```python
from build123d import *

# Parameters (mm, degrees)
BOSS_EXTRUDE1_DEPTH = 48
CHAMFER1_SIZE       = 1
CHAMFER1_SIZE2      = 0.5
CHAMFER2_SIZE       = 0.5
CHAMFER2_SIZE2      = 1.5
CHAMFER3_SIZE       = 0.5
CHAMFER3_SIZE2      = 2.5
CHAMFER4_SIZE       = 2.5
CHAMFER4_SIZE2      = 0.5
CHAMFER5_SIZE       = 4
CHAMFER5_SIZE2      = 3.356398525
CHAMFER6_SIZE       = 4
CHAMFER6_SIZE2      = 3.356398525
FILLET1_R           = 2


with BuildPart() as part:
    # Sketch1 → Boss-Extrude1 (new body)
    with BuildSketch(Plane(origin=(0, 0, 0), x_dir=(1, 0, 0), z_dir=(0, 1, 0))):
        Polygon((-7.5, 2.25), (7.5, 2.25), (7.5, -2.25), (2.45, -2.25), (2.45, -6.75), (2.05, -6.75), (2.05, -3.75), (-2.05, -3.75), (-2.05, -6.75), (-2.45, -6.75), (-2.45, -2.25), (-7.5, -2.25), align=None)
    extrude(amount=BOSS_EXTRUDE1_DEPTH)

    # Chamfer1
    chamfer1_edges = [part.edges().sort_by_distance(p)[0] for p in [
        (-2.05, 24, 3.75),
    ]]
    chamfer1_side = [part.faces().sort_by_distance(p)[0] for p in [
        (-2.05, 24, 5.25),
    ]]
    chamfer(chamfer1_edges, length=CHAMFER1_SIZE, length2=CHAMFER1_SIZE2, reference=chamfer1_side[0])

    # Chamfer2
    chamfer2_edges = [part.edges().sort_by_distance(p)[0] for p in [
        (2.05, 24, 3.75),
    ]]
    chamfer2_side = [part.faces().sort_by_distance(p)[0] for p in [
        (0.25, 24, 3.75),
    ]]
    chamfer(chamfer2_edges, length=CHAMFER2_SIZE, length2=CHAMFER2_SIZE2, reference=chamfer2_side[0])

    # Chamfer3
    chamfer3_edges = [part.edges().sort_by_distance(p)[0] for p in [
        (-2.45, 24, 2.25),
    ]]
    chamfer3_side = [part.faces().sort_by_distance(p)[0] for p in [
        (-4.975, 24, 2.25),
    ]]
    chamfer(chamfer3_edges, length=CHAMFER3_SIZE, length2=CHAMFER3_SIZE2, reference=chamfer3_side[0])

    # Chamfer4
    chamfer4_edges = [part.edges().sort_by_distance(p)[0] for p in [
        (2.45, 24, 2.25),
    ]]
    chamfer4_side = [part.faces().sort_by_distance(p)[0] for p in [
        (2.45, 24, 4.5),
    ]]
    chamfer(chamfer4_edges, length=CHAMFER4_SIZE, length2=CHAMFER4_SIZE2, reference=chamfer4_side[0])

    # Chamfer5
    chamfer5_edges = [part.edges().sort_by_distance(p)[0] for p in [
        (-7.5, 24, 2.25),
    ]]
    chamfer5_side = [part.faces().sort_by_distance(p)[0] for p in [
        (-7.5, 24, 0),
    ]]
    chamfer(chamfer5_edges, length=CHAMFER5_SIZE, length2=CHAMFER5_SIZE2, reference=chamfer5_side[0])

    # Chamfer6
    chamfer6_edges = [part.edges().sort_by_distance(p)[0] for p in [
        (7.5, 24, 2.25),
    ]]
    chamfer6_side = [part.faces().sort_by_distance(p)[0] for p in [
        (7.5, 24, 0),
    ]]
    chamfer(chamfer6_edges, length=CHAMFER6_SIZE, length2=CHAMFER6_SIZE2, reference=chamfer6_side[0])

    # Fillet1
    fillet1_edges = [part.edges().sort_by_distance(p)[0] for p in [
        (-2.25, 0, 6.75),
        (2.25, 0, 6.75),
        (-2.25, 48, 6.75),
        (2.25, 48, 6.75),
    ]]
    fillet(fillet1_edges, radius=FILLET1_R)


solid = part.part
```
Design review of the part built by this model. Coordinates are the model's own, in mm. A direction names the side the tool comes from. Give positions to 0.01 mm unless a question says otherwise; leave off trailing zeros. Write each loop counter-clockwise with the first axis right and the second up, starting at its lowest first coordinate (ties: lowest second). Pieces come first, ordered by that corner, then holes. Notation, with made-up numbers: (7, 49.25) -> (30, 49.25) arc R33 ccw to (30, 83.25) -> close; hole circle Ø11 at (77, 72). An arc over 180 degrees is marked (long way). Answer in a Markdown table with one row per item.
(1) Consider section A-A (z = 6). State the section outline as (x, y) points, then the cut area to 3 significant figures.
Results:
| item | result |
|---|---|
| outline | (-2.45, 0.44) -> (-2.05, 0.44) -> (-2.05, 47.56) -> (-2.45, 47.56) -> close; (2.05, 0.44) -> (2.45, 0.44) -> (2.45, 47.56) -> (2.05, 47.56) -> close |
| area | 37.7 mm2 |
(2) Clearance check with flat-ended pins moving along their axes: pin 1 (2 mm diameter, centred on y = 5, z = 1.5, fed in from +X); pin 2 (1 mm diameter, centred on y = 24.5, z = 6, fed in from +X); pin 3 (1 mm diameter, centred on x = 3.5, y = 21.5, fed in from +Z). State where each tip first meets the part, or that it passes through.
Results:
| item | result |
|---|---|
| pin 1 | x = 5.61 |
| pin 2 | x = 2.45 |
| pin 3 | z = 2.25 |
(3) Consider section D-D (z = 0). State the section outline as (x, y) points.
Results:
| item | result |
|---|---|
| outline | (-6.03, 0) -> (6.03, 0) -> (6.03, 48) -> (-6.03, 48) -> close |
(4) Consider section B-B (y = 22). State the section outline as (x, z) points, then the cut area to 3 significant figures.
Results:
| item | result |
|---|---|
| outline | (-7.5, -2.25) -> (7.5, -2.25) -> (7.5, -1.75) -> (4.14, 2.25) -> (2.95, 2.25) -> (2.45, 4.75) -> (2.45, 6.75) -> (2.05, 6.75) -> (2.05, 5.25) -> (1.55, 3.75) -> (-1.55, 3.75) -> (-2.05, 4.75) -> (-2.05, 6.75) -> (-2.45, 6.75) -> (-2.45, 4.75) -> (-2.95, 2.25) -> (-4.14, 2.25) -> (-7.5, -1.75) -> close |
| area | 65.7 mm2 |
(5) To check wall thickness, follow probe 1 along X at (y, z) = (8, 6); probe 2 along Z at (x, y) = (-3, 31.5); probe 3 along X at (y, z) = (6, 4.75). State the ranges of each line that lie inside material, in increasing order.
Results:
| item | result |
|---|---|
| probe 1 | -2.45 to -2.05, 2.05 to 2.45 |
| probe 2 | -2.25 to 2.25 |
| probe 3 | -2.45 to -2.05, 1.88 to 2.45 |
(6) Mouldability with a two-part tool opening along X and no side actions: class faces 1 (the flat face through (2.7, 23.7, 3.5)), 2 (the flat face through (0, 48, 0)), 3 (the flat face through (1.8, 23.7, 4.5)) as +X half, -X half, draft (parallel to the pull), parting line (faces both ways), or undercut.
Results:
| item | result |
|---|---|
| face 1 | +X half |
| face 2 | draft |
| face 3 | undercut |
(7) For faces 4 (the flat face through (2.45, 24, 6)), 5 (the flat face through (2.05, 24, 6)), 6 (the flat face through (-3.5, 23.7, 2.25)), list the 3-axis set-ups (+Z, -Z, +X, -X, +Y, -Y) from which the entire face can be reached by the end or side of a thin tool; tool diameter is ignored.
Results:
| item | result |
|---|---|
| face 4 | +Z, +X, +Y, -Y |
| face 5 | +Z, +Y, -Y |
| face 6 | +Z, -X, +Y, -Y |
(8) Consider section C-C (x = -5.75). State the section outline as (y, z) points, then the cut area to 3 significant figures.
Results:
| item | result |
|---|---|
| outline | (0, -2.25) -> (48, -2.25) -> (48, 0.34) -> (0, 0.34) -> close |
| area | 124 mm2 |
